Input: part model. Units: mm. Frame: model coordinates. Face numbers are marked on the shaded views. Round coordinates to 2 decimals unless told otherwise and drop trailing zeros. Write each loop counter-clockwise with the first axis right and the second up, starting at its lowest first coordinate (ties: lowest second). Pieces come first, ordered by that corner, then holes. Notation, with made-up numbers: (-3, 57.25) -> (9, 57.25) arc R23 ccw to (9, 82.25) -> close; hole circle Ø10 at (-18.75, -9.75). An arc over 180 degrees is marked (long way). Write item = value, one per line.
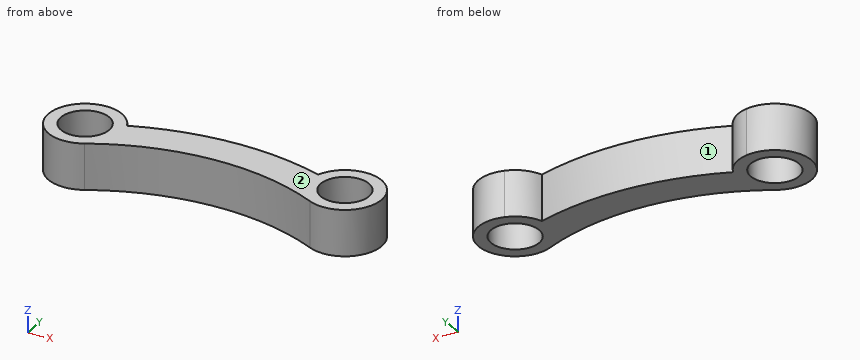
```python
from build123d import *

# Parameters (mm, degrees)
BOSS_EXTRUDE1_DEPTH = 5
SKETCH2_R           = 1.5
CUT_EXTRUDE1_DEPTH  = 3
BOSS_EXTRUDE2_DEPTH = 5
SKETCH4_R           = 2.625
CUT_EXTRUDE2_DEPTH  = 34.097061453
CUT_EXTRUDE3_DEPTH  = 34.097061453
BOSS_EXTRUDE3_DEPTH = 5


with BuildPart() as part:
    # Sketch1 → Boss-Extrude1 (new body)
    with BuildSketch(Plane.XY):
        with BuildLine():
            ThreePointArc((-26.738194812, 2.158204732), (-30.234084304, -1.121992567), (-25.515357454, -0.276679267))
            ThreePointArc((-25.515357454, -0.276679267), (-19.880574881, 1.510931441), (-14, 2.115220905))
            ThreePointArc((-14, 2.115220905), (-8.119425119, 1.510931441), (-2.484642546, -0.276679267))
            ThreePointArc((-2.484642546, -0.276679267), (2.234084304, -1.121992567), (-1.261805188, 2.158204732))
            ThreePointArc((-1.261805188, 2.158204732), (-7.461545448, 4.366267273), (-14, 5.115220905))
            ThreePointArc((-14, 5.115220905), (-20.538454552, 4.366267273), (-26.738194812, 2.158204732))
        make_face()
    extrude(amount=BOSS_EXTRUDE1_DEPTH)

    # Sketch2 → Cut-Extrude1 (cut)
    with BuildSketch(Plane.XY.offset(5)):
        with Locations((-28, 0)):
            Circle(SKETCH2_R)
        Circle(SKETCH2_R)
    extrude(amount=-CUT_EXTRUDE1_DEPTH, mode=Mode.SUBTRACT)

    # Sketch3 → Boss-Extrude2 (add, through all)
    with BuildSketch(Plane.XY.offset(5)):
        with BuildLine():
            ThreePointArc((-27.059016708, 3.887743619), (-31.451726366, -2.021283032), (-24.149017572, -1.081635031))
            ThreePointArc((-24.149017572, -1.081635031), (-14, 0.848451211), (-3.850982428, -1.081635031))
            ThreePointArc((-3.850982428, -1.081635031), (3.451726366, -2.021283032), (-0.940983292, 3.887743619))
            ThreePointArc((-0.940983292, 3.887743619), (-13.167819997, 6.801577419), (-25.534946827, 4.556552431))
            ThreePointArc((-25.534946827, 4.556552431), (-26.301527828, 4.232507508), (-27.059016708, 3.887743619))
        make_face()
    extrude(amount=-BOSS_EXTRUDE2_DEPTH)

    # Sketch4 → Cut-Extrude2 (cut, through all)
    with BuildSketch(Plane.XY.offset(5)):
        with Locations((-28, 0)):
            Circle(SKETCH4_R)
        Circle(SKETCH4_R)
    extrude(amount=-CUT_EXTRUDE2_DEPTH, mode=Mode.SUBTRACT)

    # Sketch5 → Cut-Extrude3 (cut, through all)
    with BuildSketch(Plane.XY.offset(5)):
        with BuildLine():
            Line((-14.205977149, 10.740702715), (-0.940983292, 3.887743619))
            ThreePointArc((-0.940983292, 3.887743619), (-14, 6.812890489), (-27.059016708, 3.887743619))
            Line((-27.059016708, 3.887743619), (-14.205977149, 10.740702715))
        make_face()
        with BuildLine():
            ThreePointArc((-0.940983292, 3.887743619), (-14, 6.812890489), (-27.059016708, 3.887743619))
            ThreePointArc((-27.059016708, 3.887743619), (-25.390156506, 3.031289649), (-24.295234779, 1.50821572))
            ThreePointArc((-24.295234779, 1.50821572), (-14, 3.322200059), (-3.704765221, 1.50821572))
            ThreePointArc((-3.704765221, 1.50821572), (-2.609843494, 3.031289649), (-0.940983292, 3.887743619))
        make_face()
    extrude(amount=-CUT_EXTRUDE3_DEPTH, mode=Mode.SUBTRACT)

    # Sketch7 → Boss-Extrude3 (add, through all)
    with BuildSketch(Plane.XY.offset(5)):
        with BuildLine():
            Line((-26.14792778, -3.545395393), (-24.177787081, 0.278127161))
            Line((-24.177787081, 0.278127161), (-14.756553685, 2.142998553))
            Line((-14.756553685, 2.142998553), (-4.34233682, 0.278127161))
            Line((-4.34233682, 0.278127161), (-2.53651725, -2.31550038))
            Line((-2.53651725, -2.31550038), (-1.85207222, -3.545395393))
            ThreePointArc((-1.85207222, -3.545395393), (-14, -0.563598098), (-26.14792778, -3.545395393))
        make_face()
    extrude(amount=-BOSS_EXTRUDE3_DEPTH)


solid = part.part
```
1) Cut plane A-A (x = 0). Return the cut outline in (y, z) (3 decimals), and give its area (4 significant figures).
Solutions:
outline = (-4, 0) -> (-2.625, 0) -> (-2.625, 5) -> (-4, 5) -> close; (2.625, 0) -> (4, 0) -> (4, 5) -> (2.625, 5) -> close
area = 13.75 mm^2
2) Draft query along X for the marked faces 1 and 2. Return one class per face: +X half, -X half, draft (parallel to the pull), parting line (faces both ways), or undercut.
Solutions:
face_1 = undercut
face_2 = draft
3) Line query: L1, parallel to Y at x = 0, z = 2.8 (3 decimals); L2, parallel to X at y = 0.5, z = 1.4; L3, parallel to X at y = -3.5, z = 1.1. Output: solid intervals per line, ascending. Write a range as from..to.
Solutions:
L1 = -4..-2.625, 2.625..4
L2 = -31.97..-30.58, -25.42..-2.58, 2.58..3.97
L3 = -29.94..-26.06, -1.94..1.94
4) Cut plane B-B (z = 2.35). Return the cut outline in (x, y) (3 decimals).
Solutions:
outline = (-26.148, -3.545) arc R26.236 cw to (-1.852, -3.545) arc R4 ccw (long way) to (-3.705, 1.508) arc R30.122 ccw to (-24.295, 1.508) arc R4 ccw (long way) to start; hole circle Ø5.25 at (-28, 0); hole circle Ø5.25 at (0, 0)
5) Cut plane C-C (y = 0). Return the cut outline in (x, z) (3 decimals).
Solutions:
outline = (-32, 0) -> (-30.625, 0) -> (-30.625, 5) -> (-32, 5) -> close; (-25.375, 0) -> (-2.625, 0) -> (-2.625, 5) -> (-25.375, 5) -> close; (2.625, 0) -> (4, 0) -> (4, 5) -> (2.625, 5) -> close
6) First-contact query: P1, Ø1, axis at y = 2, z = 0.5, coming from the +X side. Flat tip, straight axial feed; report the tip coordinate or a pass-through.
Solutions:
P1 = 3.71
7) Cut plane D-D (y = 2). Return the cut outline in (x, z), and give its area (3 significant figures).
Solutions:
outline = (-31.46, 0) -> (-29.7, 0) -> (-29.7, 5) -> (-31.46, 5) -> close; (-26.3, 0) -> (-24.54, 0) -> (-24.54, 5) -> (-26.3, 5) -> close; (-22.83, 0) -> (-5.17, 0) -> (-5.17, 5) -> (-22.83, 5) -> close; (-3.46, 0) -> (-1.7, 0) -> (-1.7, 5) -> (-3.46, 5) -> close; (1.7, 0) -> (3.46, 0) -> (3.46, 5) -> (1.7, 5) -> close
area = 124 mm^2
